Source: CAD feature listing. Evaluate the final solid. Frame: model axes, mm. A direction names the side the tool comes from. Coordinates: 2 decimals unless noted, no trailing zeros. Order: outer loops, then holes, each group sorted by start corner. A loop starts at its lowest first (then second) coordinate and runs counter-clockwise, first axis right, second up.
```python
from build123d import *


with BuildPart() as part:
    # Sketch1 → Revolve1 (revolve)
    with BuildSketch(Plane.XY, mode=Mode.PRIVATE) as revolve1_sk:
        with BuildLine():
            Line((0, 65), (0, 142.5))
            Line((0, 142.5), (24, 142.5))
            Line((24, 142.5), (24, 80))
            Line((24, 80), (34.398449785, 80))
            ThreePointArc((34.398449785, 80), (41.732480398, 80.910276815), (48.621444476, 83.585867002))
            Line((48.621444476, 83.585867002), (130.980482924, 127.933041551))
            ThreePointArc((130.980482924, 127.933041551), (153.943696517, 136.851675508), (178.390465228, 139.885931559))
            Line((178.390465228, 139.885931559), (183.05792065, 139.885931559))
            ThreePointArc((183.05792065, 139.885931559), (193.313652481, 137.056253763), (200.667342649, 129.36792802))
            Line((200.667342649, 129.36792802), (218.75476257, 95.777005309))
            ThreePointArc((218.75476257, 95.777005309), (229.785297821, 84.244516693), (245.168895567, 80))
            Line((245.168895567, 80), (276, 80))
            Line((276, 80), (276, 142.5))
            Line((276, 142.5), (300, 142.5))
            Line((300, 142.5), (300, 65))
            Line((300, 65), (0, 65))
        make_face()
    revolve(revolve1_sk.sketch.rotate(Axis((0, 0, 0), (1, 0, 0)), 90), axis=Axis((0, 0, 0), (1, 0, 0)))


solid = part.part
```
1. Section query C-C on x = 42.5. Return loops of the section in (y, z), plus the area to 3 significant figures.
Findings:
outline: circle Ø162.23 at (0, 0); hole circle Ø130 at (0, 0)
area: 7,400 mm2
2. Ray query, line 1 (X direction, y = 93, z = -37.5); line 2 (X direction, y = 93, z = 44); line 3 (X direction, y = -118.5, z = -75.5). Return the intervals inside material, ascending.
Findings:
line 1: x = 0 to 24, 79.62 to 216.33, 276 to 300
line 2: x = 0 to 24, 84.46 to 214.93, 276 to 300
line 3: x = 0 to 24, 276 to 300
3. Section query D-D on x = 117.5. Return loops of the section in (y, z).
Findings:
outline: circle Ø241.35 at (0, 0); hole circle Ø130 at (0, 0)
4. Access query for faces 4 (the face through (260.8, -3.517, -79.923)), 5 (the face through (300, 61, 30)). Directions: +Z, -Z, +X, -X, +Y, -Y. A direction counts if a zero-diameter tool reaches every point of the face in a straight line with its end or side. Return the directions, or none.
Findings:
face 4: none
face 5: +Z, -Z, +X, +Y, -Y
5. Pin query (flat end, axial travel): P1, Ø10, axis at x = 119.5, z = -95.5, coming from the +Y side; P2, Ø6, axis at x = 213, y = 29, coming from the +Z side; P3, Ø12, axis at x = 147.5, y = -61, coming from the -Z side. Return the tip coordinate at first contact, or that it passes through.
Findings:
P1: stops at y = 82.75
P2: stops at z = 108.27
P3: stops at z = -123.95
6. Draft query along Y for faces 1 (the face through (147.9, -19.52, 62)), 2 (the face through (217.877, 59.271, -77.3)), 3 (the face through (276, 61, -61)). Return one class per face: released by +Y, released by -Y, zero draft, split by the parting line, or undercut.
Findings:
face 1: undercut
face 2: split by the parting line
face 3: zero draft
7. Section query A-A on z = -112. Count the separate pieces of the cut face and the enclosed holes in it, plus the area to 3 significant figures.
Findings:
separate pieces: 3
enclosed holes: 0
area: 22,500 mm2
